Input: part model. Units: mm. Frame: model coordinates. A direction names the side the tool comes from. Coordinates: 2 decimals unless noted, no trailing zeros. Loops run counter-clockwise (first coordinate to the right, second up) from the corner with the lowest first, then second, coordinate; pieces in that order, holes last. Notation, with made-up numbers: (21.25, -23.75) - (75.25, -23.75) arc R11 ccw to (75.25, -15.75) - close; hole circle Ø5 at (3.5, 67). An arc over 180 degrees is marked (long way). Use one line per item in the form item = value.
from build123d import *

# Parameters (mm, degrees)
SKETCH1_W                                            = 503
SKETCH1_H                                            = 130
BOSS_EXTRUDE1_DEPTH                                  = 7
SKETCH2_W                                            = 363
SKETCH2_H                                            = 60
CUT_EXTRUDE1_DEPTH                                   = 261.140827246
M5_TAPPED_HOLE1_D                                    = 4.2
HOLE_SIZE_PER_SOCKET_HEAD_CAP_SCREW_TYPE_D           = 6.6
HOLE_SIZE_PER_SOCKET_HEAD_CAP_SCREW_TYPE_CBORE_D     = 11
HOLE_SIZE_PER_SOCKET_HEAD_CAP_SCREW_TYPE_CBORE_DEPTH = 6.8
M8_CLEARANCE_HOLE1_D                                 = 9
HOLE_SIZE_PER_SOCKET_HEAD_CAP_SCREW_2_D              = 6.6
HOLE_SIZE_PER_SOCKET_HEAD_CAP_SCREW_2_CBORE_D        = 11
HOLE_SIZE_PER_SOCKET_HEAD_CAP_SCREW_2_CBORE_DEPTH    = 6.8
FILLET2_R                                            = 20
CHAMFER1_SIZE                                        = 1
SKETCH12_W                                           = 15
SKETCH12_H                                           = 95
BOSS_EXTRUDE2_DEPTH                                  = 14
SKETCH13_R                                           = 5
CUT_EXTRUDE2_DEPTH                                   = 10
M5_CLEARANCE_HOLE1_D                                 = 5.5
FILLET3_R                                            = 5
CHAMFER2_SIZE                                        = 1


with BuildPart() as part:
    # Sketch1 → Boss-Extrude1 (new, symmetric)
    with BuildSketch(Plane(origin=(0, 0, 0), x_dir=(1, 0, 0), z_dir=(0, 1, 0))):
        Rectangle(SKETCH1_W, SKETCH1_H)
    extrude(amount=BOSS_EXTRUDE1_DEPTH, both=True)

    # Sketch2 → Cut-Extrude1 (cut, through all)
    with BuildSketch(Plane(origin=(0, 7, 0), x_dir=(1, 0, 0), z_dir=(0, 1, 0))):
        with Locations((-70, -35)):
            Rectangle(SKETCH2_W, SKETCH2_H)
    extrude(amount=-CUT_EXTRUDE1_DEPTH, mode=Mode.SUBTRACT)

    # M5 Tapped Hole1 (through all)
    with Locations(Plane(origin=(0, 7, 0), x_dir=(1, 0, 0), z_dir=(0, 1, 0))):
        with Locations((201.5, -55), (201.5, -27), (201.5, 1)):
            Hole(M5_TAPPED_HOLE1_D / 2)

    # Hole Size per Socket Head Cap Screw Type (through all)
    with Locations(Plane(origin=(0, -7, 0), x_dir=(-1, 0, 0), z_dir=(0, -1, 0))):
        with Locations((-8.5, 57), (191.5, 57), (91.5, 57)):
            CounterBoreHole(HOLE_SIZE_PER_SOCKET_HEAD_CAP_SCREW_TYPE_D / 2, HOLE_SIZE_PER_SOCKET_HEAD_CAP_SCREW_TYPE_CBORE_D / 2, HOLE_SIZE_PER_SOCKET_HEAD_CAP_SCREW_TYPE_CBORE_DEPTH)

    # M8 Clearance Hole1 (through all)
    with Locations(Plane(origin=(0, 7, 0), x_dir=(1, 0, 0), z_dir=(0, 1, 0))):
        with Locations((134.5, 7.5), (244.5, -42.5), (134.5, -42.5), (244.5, 7.5)):
            Hole(M8_CLEARANCE_HOLE1_D / 2)

    # Hole Size per Socket Head Cap Screw  2 (through all)
    with Locations(Plane(origin=(0, -7, 0), x_dir=(-1, 0, 0), z_dir=(0, -1, 0))):
        with Locations((-238.5, 33), (241.5, 33), (141.5, 33), (41.5, 33), (-58.5, 33), (-158.5, 33)):
            CounterBoreHole(HOLE_SIZE_PER_SOCKET_HEAD_CAP_SCREW_2_D / 2, HOLE_SIZE_PER_SOCKET_HEAD_CAP_SCREW_2_CBORE_D / 2, HOLE_SIZE_PER_SOCKET_HEAD_CAP_SCREW_2_CBORE_DEPTH)

    # Fillet2
    fillet2_edges = [part.edges().sort_by_distance(p)[0] for p in [
        (111.5, 0, 5),
    ]]
    fillet(fillet2_edges, radius=FILLET2_R)

    # Chamfer1
    chamfer1_edges = [part.edges().sort_by_distance(p)[0] for p in [
        (111.5, 0, 65),
        (-251.5, 0, -65),
        (251.5, 0, -65),
    ]]
    chamfer(chamfer1_edges, length=CHAMFER1_SIZE)

    # Sketch12 → Boss-Extrude2 (add)
    with BuildSketch(Plane(origin=(0, 7, 0), x_dir=(1, 0, 0), z_dir=(0, 1, 0))):
        with Locations((259, -17.5)):
            Rectangle(SKETCH12_W, SKETCH12_H)
    extrude(amount=-BOSS_EXTRUDE2_DEPTH)

    # Sketch13 → Cut-Extrude2 (cut)
    with BuildSketch(Plane.XZ.offset(7)):
        with Locations(Location((122.5, 53, 0), (0, 0, 270))):
            Circle(SKETCH13_R)
        with Locations(Location((256.5, 53, 0), (0, 0, 90))):
            Circle(SKETCH13_R)
        with Locations(Location((256.5, -18, 0), (0, 0, 270))):
            Circle(SKETCH13_R)
        with Locations(Location((122.5, -18, 0), (0, 0, 90))):
            Circle(SKETCH13_R)
    extrude(amount=-CUT_EXTRUDE2_DEPTH, mode=Mode.SUBTRACT)

    # M5 Clearance Hole1 (through all)
    with Locations(Plane(origin=(0, 7, 0), x_dir=(1, 0, 0), z_dir=(0, 1, 0))):
        with Locations((122.5, 18), (122.5, -53), (256.5, -53), (256.5, 18)):
            Hole(M5_CLEARANCE_HOLE1_D / 2)

    # Fillet3
    fillet3_edges = [part.edges().sort_by_distance(p)[0] for p in [
        (251.5, 0, -30),
    ]]
    fillet(fillet3_edges, radius=FILLET3_R)

    # Chamfer2
    chamfer2_edges = [part.edges().sort_by_distance(p)[0] for p in [
        (266.5, 0, 65),
        (266.5, 0, -30),
    ]]
    chamfer(chamfer2_edges, length=CHAMFER2_SIZE)


solid = part.part
Q1. Ray query, line 1 along X through (y, z) = (2.5, -57); line 2 along Z through (x, y) = (201.5, 2); line 3 along Z through (x, y) = (256.5, 6.15). Return the intervals inside material, ascending. Write a range as [from, to].
Check values:
line_1 = [-251.5, -194.8], [-188.2, -94.8], [-88.2, 5.2], [11.8, 251.5]
line_2 = [-65, -3.1], [1.1, 24.9], [29.1, 52.9], [57.1, 65]
line_3 = [-30, -20.75], [-15.25, 50.25], [55.75, 65]
Q2. Pull-direction query (X, two-part tool) for faces 1 (the cylindrical face through (9.216, -3.648, -62.453)), 2 (the flat face through (61, 7, -15)), 3 (the cylindrical face through (105.486, -0.098, 10.703)); classes: pulls with the +X half, pulls with the -X half, needs draft (parallel to the pull), parting line crosses it, or undercut.
Check values:
face_1 = undercut
face_2 = needs draft
face_3 = pulls with the -X half
Q3. Set-up query: faces 4 (the flat face through (-41, -0.2, -29)), 5 (the cylindrical face through (135.48, -0.1, 46.89)), 6 (the flat face through (111.5, 0, 45)). Return all of +Z, -Z, +X, -X, +Y, -Y with unobstructed straight access to the full face (end or side cutting, diameter ignored); none if empty.
Check values:
face_4 = -Y
face_5 = +Y, -Y
face_6 = +Z, -X, +Y, -Y
Q4. Cut plane B-B, the plane y = -4.25. Give the number of separate pieces and of enclosed holes in the cut face, then the cut area to 3 significant figures.
Check values:
separate_pieces = 1
enclosed_holes = 20
area = 43,700 mm²
Q5. First-contact query: P1, Ø1, axis at x = 81, y = -0.5, coming from the +Z side; P2, Ø7, axis at x = 259.5, y = -2, coming from the -Z side; P3, Ø3.5, axis at x = 156.5, z = -35, coming from the -Y side. Flat tips, straight axial feed; report the tip coordinate or a pass-through.
Check values:
P1 = 5
P2 = -30.03
P3 = -0.2
Q6. Cut plane A-A, the plane x = -211. Return loops of the section in (y, z).
Check values:
outline = (-7, -65) - (7, -65) - (7, 5) - (-7, 5) - close
